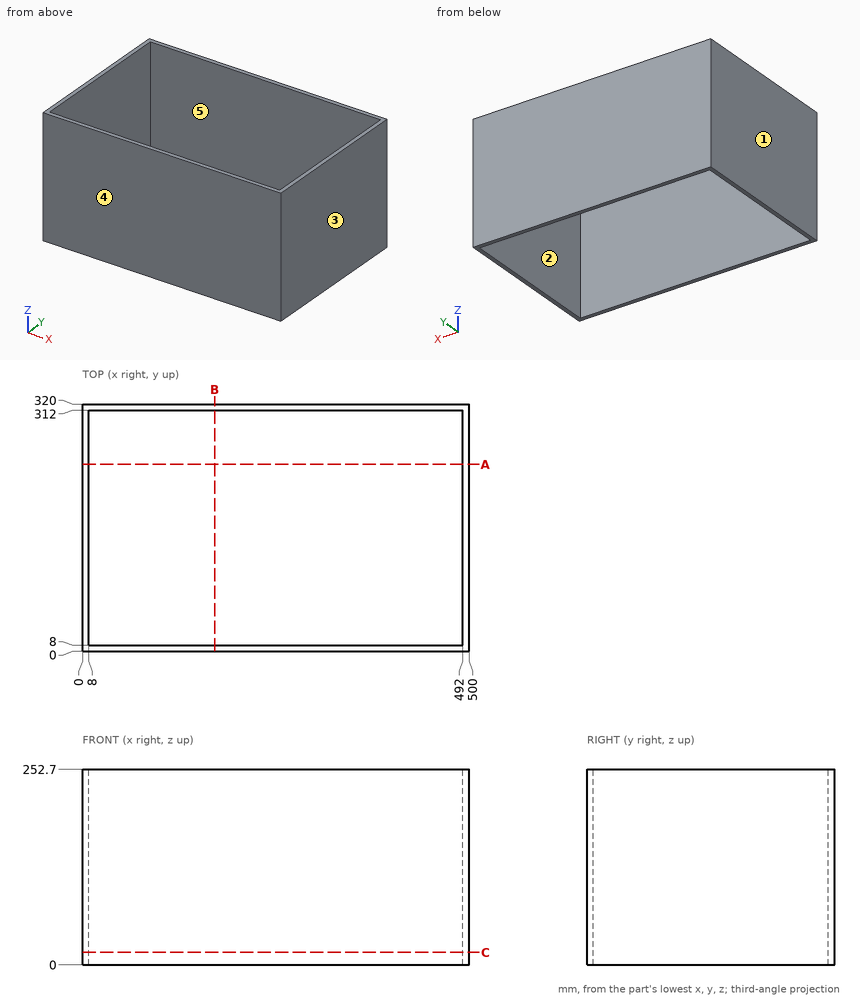
Geometry check sheet. Reference: drawing and pictorial views, mm from the part's lowest x, y, z. A direction names the side the tool comes from. Give positions to 0.01 mm unless a question says otherwise; leave off trailing zeros. Order: outer loops, then holes, each group sorted by start corner. A loop starts at its lowest first (then second) coordinate and runs counter-clockwise, first axis right, second up. Notation, with made-up numbers: M 74,-20 L 128,-20 A26 cw 128,11 Z; hole C -25,30.25 d7. An arc over 180 degrees is marked long. Answer in a Markdown table with one row per item.
1) Cross-section at C-C, the plane z = 16. Enter the section's corners in (x, y).
Filled sheet:
| item | result |
|---|---|
| outline | M 0,0 L 500,0 L 500,320 L 0,320 Z; hole M 8,8 L 492,8 L 492,312 L 8,312 Z |
2) Cross-section at A-A, the plane y = 242. Enter the section's corners in (x, z), plus the area to 3 significant figures.
Filled sheet:
| item | result |
|---|---|
| outline | M 0,0 L 8,0 L 8,252.7 L 0,252.7 Z; M 492,0 L 500,0 L 500,252.7 L 492,252.7 Z |
| area | 4,040 mm2 |
3) Cross-section at B-B, the plane x = 171. Enter the section's corners in (y, z), plus the area to 3 significant figures.
Filled sheet:
| item | result |
|---|---|
| outline | M 0,0 L 8,0 L 8,252.7 L 0,252.7 Z; M 312,0 L 320,0 L 320,252.7 L 312,252.7 Z |
| area | 4,040 mm2 |
4) Thickness scan on L1, parallel to X at y = 230, z = 217; L2, parallel to Y at x = 104, z = 143. Record the ranges inside material, lowest first. Write a range as [from, to].
Filled sheet:
| item | result |
|---|---|
| L1 | x = [0, 8], [492, 500] |
| L2 | y = [0, 8], [312, 320] |
5) Access from +Z, -Z, +X, -X, +Y, -Y to the whole of each face (thin tool, end or side, straight path). Record for the marked faces 1 and 2.
Filled sheet:
| item | result |
|---|---|
| face 1 | +Z, -Z, -X, +Y, -Y |
| face 2 | +Z, -Z |
6) Release check for a two-part mould opening along X. For the marked faces 3, 4 and 5 record: +X half, -X half, draft (parallel to the pull), parting line (faces both ways), or undercut.
Filled sheet:
| item | result |
|---|---|
| face 3 | +X half |
| face 4 | draft |
| face 5 | undercut |
